Verification items for the finished model (mm, model axes). Face numbers are marked on the shaded views. A direction names the side the tool comes from. Coordinates: 2 decimals unless noted, no trailing zeros. Order: outer loops, then holes, each group sorted by start corner. A loop starts at its lowest first (then second) coordinate and runs counter-clockwise, first axis right, second up. Notation, with made-up numbers: M 43.25,80.25 L 58.25,80.25 A28 ccw 58.25,117.25 Z; hole C 0,78.5 d6. An arc over 180 degrees is marked long. Return JSON: item names as keys, results as strings. Group by question number.
Q1. Section check B-B, the plane y = 10. Enter the section's corners in (x, z), then the cut area to 4 significant figures.
Q2. Section check A-A, the plane x = 2. Enter the section's corners in (y, z).
Q3. Access from +Z, -Z, +X, -X, +Y, -Y to the whole of each face (thin tool, end or side, straight path). Record for the marked faces 1, 2, 3 and 4.
Q4. Go/stop test with flat-tipped pins: pin 1 Ø1 at (x, z) = (-2.5, -1) entering from -Y; pin 2 Ø8 at (y, z) = (15, 13.5) entering from -X; pin 3 Ø6 at (y, z) = (12, 3.5) entering from +X; pin 4 Ø9 at (x, y) = (3.5, 6.5) entering from -Z. Record where each tip stops, or that it passes through.
Q5. Section check D-D, the plane x = -10. Enter the section's corners in (y, z), then the cut area to 3 significant figures.
Q6. Thickness scan on probe 1 along Y at (x, z) = (7.5, 14.25); probe 2 along Z at (x, y) = (-8, 16.75); probe 3 along X at (y, z) = (3, 8). Record the ranges inside material, lowest first.
Q7. Section check C-C, the plane z = 5. Enter the section's corners in (x, y).
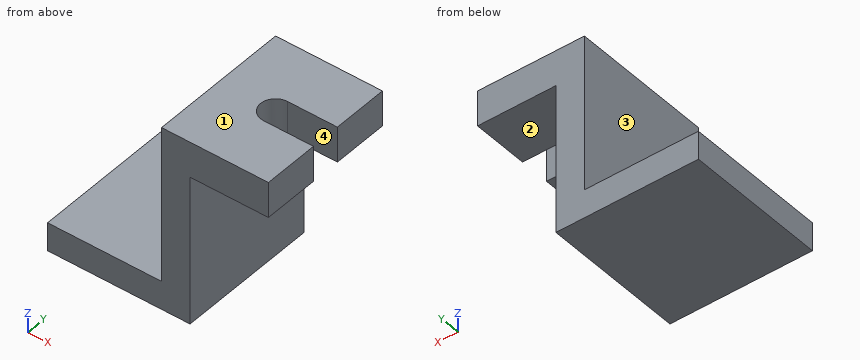
from build123d import *

# Parameters (mm, degrees)
SKETCH1_W           = 16
SKETCH1_H           = 4
SKETCH1_W_2         = 4
SKETCH1_H_2         = 17
SKETCH1_H_3         = 5
SKETCH1_W_3         = 11
BOSS_EXTRUDE1_DEPTH = 20
CUT_EXTRUDE1_DEPTH  = 15


with BuildPart() as part:
    # Sketch1 → Boss-Extrude1 (new body)
    with BuildSketch(Plane(origin=(0, 0, 0), x_dir=(1, 0, 0), z_dir=(0, 1, 0))):
        with Locations((-14.574257426, 6.653465347)):
            Rectangle(SKETCH1_W, SKETCH1_H)
        with Locations((-4.574257426, 6.653465347)):
            Rectangle(SKETCH1_W_2, SKETCH1_H)
        with Locations((-4.574257426, -3.846534653)):
            Rectangle(SKETCH1_W_2, SKETCH1_H_2)
        with Locations((-4.574257426, -14.846534653)):
            Rectangle(SKETCH1_W_2, SKETCH1_H_3)
        with Locations((2.925742574, -14.846534653)):
            Rectangle(SKETCH1_W_3, SKETCH1_H_3)
    extrude(amount=BOSS_EXTRUDE1_DEPTH)

    # Sketch2 → Cut-Extrude1 (cut)
    with BuildSketch(Plane(origin=(0, 0, 12.346534653), x_dir=(-1, 0, 0), z_dir=(0, 0, -1))):
        with BuildLine():
            Line((-5.425742574, 7.9), (-8.841676891, 7.9))
            Line((-8.841676891, 7.9), (-8.841676891, 11.852277474))
            Line((-8.841676891, 11.852277474), (-8.841676891, 12.1))
            Line((-8.841676891, 12.1), (-5.425742574, 12.1))
            Line((-5.425742574, 12.1), (-1.425742574, 12.1))
            ThreePointArc((-1.425742574, 12.1), (0.674257426, 10), (-1.425742574, 7.9))
            Line((-1.425742574, 7.9), (-5.425742574, 7.9))
        make_face()
    extrude(amount=-CUT_EXTRUDE1_DEPTH, mode=Mode.SUBTRACT)


solid = part.part
Numbers:
{
 "1": {"outline": "M -22.57,-8.65 L -2.57,-8.65 L -2.57,12.35 L -0.67,12.35 L -0.67,17.35 L -6.57,17.35 L -6.57,-4.65 L -22.57,-4.65 Z", "area": "177.5 mm2"},
 "2": {"outline": "M 0,12.35 L 7.9,12.35 L 7.9,17.35 L 0,17.35 Z; M 12.1,12.35 L 20,12.35 L 20,17.35 L 12.1,17.35 Z"},
 "3": {"face 1": "+Z, +X, -X, +Y, -Y", "face 2": "-Z, +X, +Y, -Y", "face 3": "+Z, -X, +Y, -Y", "face 4": "+Z, -Z, +X"},
 "4": {"pin 1": "stops at y = 0", "pin 2": "stops at x = -6.57", "pin 3": "stops at x = -2.57", "pin 4": "stops at z = 12.35"},
 "5": {"outline": "M 0,-8.65 L 20,-8.65 L 20,-4.65 L 0,-4.65 Z", "area": "80.0 mm2"},
 "6": {"probe 1": "y = 0 to 7.9, 12.1 to 20", "probe 2": "z = -8.65 to -4.65", "probe 3": "x = -6.57 to -2.57"},
 "7": {"outline": "M -6.57,0 L -2.57,0 L -2.57,20 L -6.57,20 Z"}
}
